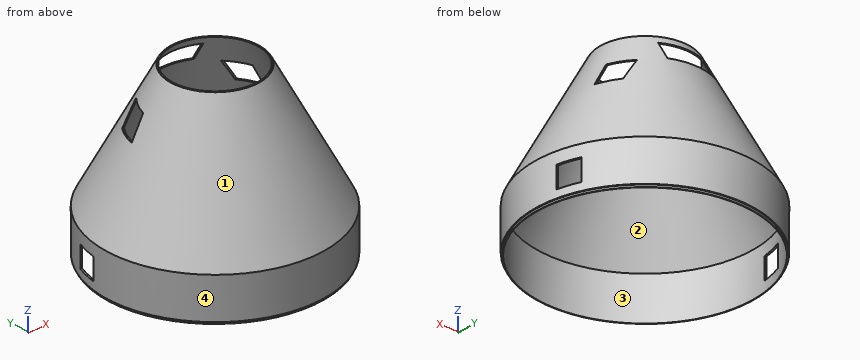
from build123d import *

# Parameters (mm, degrees)
SKETCH2_R           = 254
SKETCH2_R_2         = 250
BOSS_EXTRUDE1_DEPTH = 100
SKETCH7_W           = 50
SKETCH7_H           = 50
CUT_EXTRUDE3_DEPTH  = 500
SKETCH8_R           = 254
SKETCH8_R_2         = 251.5
CUT_EXTRUDE4_DEPTH  = 5
CUT_EXTRUDE5_START  = 100
SKETCH9_W           = 114.623557318
SKETCH9_H           = 40.936984757
CUT_EXTRUDE5_DEPTH  = 200


with BuildPart() as part:
    # Sketch2 → Boss-Extrude1 (new body)
    with BuildSketch(Plane.XY):
        Circle(SKETCH2_R)
        Circle(SKETCH2_R_2, mode=Mode.SUBTRACT)
    extrude(amount=BOSS_EXTRUDE1_DEPTH)

    # Sketch5 → Revolve1 (revolve)
    with BuildSketch(Plane(origin=(0, 0, 0), x_dir=(1, 0, 0), z_dir=(0, 1, 0)), mode=Mode.PRIVATE) as revolve1_sk:
        Polygon((254, -100), (103.395722574, -384), (100, -384), (250.604277426, -100), align=None)
    revolve(revolve1_sk.sketch.rotate(Axis((0, 0, 0), (0, 0, 1)), 180), axis=Axis((0, 0, 0), (0, 0, 1)))

    # Sketch7 → Cut-Extrude3 (cut, symmetric)
    with BuildSketch(Plane(origin=(0, 0, 0), x_dir=(0, 0, -1), z_dir=(1, 0, 0))):
        with Locations((-47.8, 67.9)):
            Rectangle(SKETCH7_W, SKETCH7_H)
        with Locations((-292.2, 67.9)):
            Rectangle(SKETCH7_W, SKETCH7_H)
    extrude(amount=CUT_EXTRUDE3_DEPTH, both=True, mode=Mode.SUBTRACT)

    # Sketch8 → Cut-Extrude4 (cut)
    with BuildSketch(Plane(origin=(0, 0, 0), x_dir=(-1, 0, 0), z_dir=(0, 0, -1))):
        Circle(SKETCH8_R)
        Circle(SKETCH8_R_2, mode=Mode.SUBTRACT)
    extrude(amount=-CUT_EXTRUDE4_DEPTH, mode=Mode.SUBTRACT)

    # Sketch9 → Cut-Extrude5 (cut)
    with BuildSketch(Plane(origin=(600, 66.233541641, 45.300312461), x_dir=(1, 0, 0), z_dir=(0, 1, 0)).offset(CUT_EXTRUDE5_START)):
        with Locations((-599.905010531, -300.978332918)):
            Rectangle(SKETCH9_W, SKETCH9_H)
    extrude(amount=-CUT_EXTRUDE5_DEPTH, mode=Mode.SUBTRACT)


solid = part.part
Could you check a few things on this model? Use its own coordinates, in mm. Face numbers are marked on the shaded views. A direction names the side the tool comes from. Give positions to 0.01 mm unless a question says otherwise; leave off trailing zeros. Order: outer loops, then holes, each group sorted by start corner. A loop starts at its lowest first (then second) coordinate and runs counter-clockwise, first axis right, second up. Notation, with made-up numbers: (45, 73) - (99, 73) arc R23 cw to (99, 108) - close; hole circle Ø10 at (-19.5, 11.5). An arc over 180 degrees is marked (long way). One line per item, written item: value. Start each with the question number.
1. Imagine slicing it at D-D on z = 120. List the corners of the cut face in (x, y) for me, plus the area to 3 significant figures.
2. Imagine slicing it at C-C on y = 85. Give the number of separate pieces and of enclosed holes in the cut face, plus the area to 3 significant figures.
3. Thinking about a two-plate mould opening in Y: for the marked faces 1 and 2, which applies, +Y half, -Y half, draft (parallel to the pull), parting line (faces both ways), or undercut?
4. If I drill on probe 1 along Y at (x, z) = (0, 22); probe 2 along X at (y, z) = (43, 96.5); probe 3 along Y at (x, z) = (-65, 268), over which ranges is the centre line in solid material (lowest first)?
5. Imagine slicing it at A-A on y = 0. List the corners of the cut face in (x, z) for me, plus the area to 3 significant figures.
6. For P1, Ø2, axis at x = -248.5, z = 56, coming from the +Y side; P2, Ø14.5, axis at y = 100, z = 349.5, coming from the -X side; P3, Ø2, axis at x = 129.5, y = -107.5, coming from the +Z side, each with a flat end and sliding along its axis, tell me the tip position at first contact or that it passes through.
7. Imagine slicing it at B-B on x = 0. List the corners of the cut face in (y, z) for me, plus the area to 3 significant figures.
8. For the marked faces 3 and 4, which set-ups out of +Z, -Z, +X, -X, +Y, -Y let a thin tool reach every point of the face, with its end or its side?
Values:
1. outline: circle Ø486.79 at (0, 0); hole circle Ø480 at (0, 0)
1. area: 5,160 mm²
2. separate pieces: 6
2. enclosed holes: 0
2. area: 2,310 mm²
3. face 1: parting line
3. face 2: undercut
4. probe 1: -254 to -250, 250 to 254
4. probe 2: -250.33 to -246.27, 246.27 to 250.33
4. probe 3: -151.56 to -147.86, 147.86 to 151.56
5. outline: (-254, 5) - (-251.5, 5) - (-251.5, 0) - (-250, 0) - (-250, 100) - (-250.6, 100) - (-100, 384) - (-103.4, 384) - (-254, 100) - close; (100, 384) - (250.6, 100) - (250, 100) - (250, 0) - (251.5, 0) - (251.5, 5) - (254, 5) - (254, 100) - (103.4, 384) - close
5. area: 2,700 mm²
6. P1: y = 42.9
6. P2: x = -80.64
6. P3: z = 263.48
7. outline: (-254, 5) - (-251.5, 5) - (-251.5, 0) - (-250, 0) - (-250, 100) - (-250.6, 100) - (-100, 384) - (-103.4, 384) - (-254, 100) - close; (100, 384) - (109.15, 366.75) - (112.54, 366.75) - (103.4, 384) - close; (130.86, 325.81) - (250.6, 100) - (250, 100) - (250, 0) - (251.5, 0) - (251.5, 5) - (254, 5) - (254, 100) - (134.25, 325.81) - close
7. area: 2,560 mm²
8. face 3: -Z
8. face 4: +Z, -Z
